The listing builds one solid part. Answer for the finished solid, in the listing's coordinates (mm). Face numbers are marked on the shaded views. A direction names the side the tool comes from. Round coordinates to 2 decimals unless told otherwise and drop trailing zeros. Write each loop counter-clockwise with the first axis right and the second up, starting at its lowest first coordinate (ties: lowest second). Pieces come first, ordered by that corner, then holes. Notation, with made-up numbers: (38, -28.75) - (63, -28.75) arc R15 cw to (63, -7.75) - close; hole circle Ø5 at (-40, 41). An arc over 180 degrees is marked (long way). Answer in a Markdown table with one row per item.
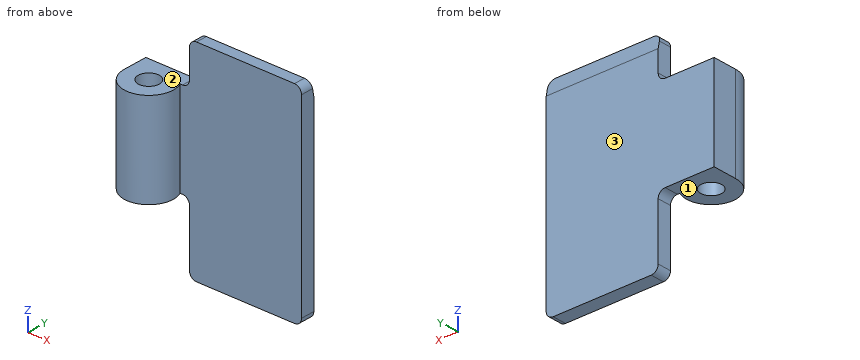
from build123d import *

# Parameters (mm, degrees)
SKETCH1_R           = 1.75
BOSS_EXTRUDE1_DEPTH = 6.7
SKETCH2_R           = 0.75
CUT_EXTRUDE1_DEPTH  = 8.142478561
SKETCH3_W           = 12
SKETCH3_H           = 6.7
BOSS_EXTRUDE2_DEPTH = 1
BOSS_EXTRUDE3_START = -6.7
BOSS_EXTRUDE3_DEPTH = 6.7
SKETCH5_W           = 8
SKETCH5_H           = 1
BOSS_EXTRUDE4_DEPTH = 3
SKETCH6_W           = 8
SKETCH6_H           = 1
BOSS_EXTRUDE5_DEPTH = 5
CHAMFER1_SIZE       = 1
CHAMFER1_SIZE2      = 0.2
FILLET1_R           = 0.5


with BuildPart() as part:
    # Sketch1 → Boss-Extrude1 (new body)
    with BuildSketch(Plane.XY):
        Circle(SKETCH1_R)
    extrude(amount=BOSS_EXTRUDE1_DEPTH)

    # Sketch2 → Cut-Extrude1 (cut, through all)
    with BuildSketch(Plane.XY.offset(6.7)):
        Circle(SKETCH2_R)
    extrude(amount=-CUT_EXTRUDE1_DEPTH, mode=Mode.SUBTRACT)

    # Sketch3 → Boss-Extrude2 (add)
    with BuildSketch(Plane(origin=(0, 1.75, 0), x_dir=(1, 0, 0), z_dir=(0, 1, 0))):
        with Locations((4.25, -3.35)):
            Rectangle(SKETCH3_W, SKETCH3_H)
    extrude(amount=-BOSS_EXTRUDE2_DEPTH)

    # Sketch4 → Boss-Extrude3 (add)
    with BuildSketch(Plane.XY.offset(6.7).offset(BOSS_EXTRUDE3_START)):
        with BuildLine():
            Line((-1.75, 0.75), (-1.75, 0))
            ThreePointArc((-1.75, 0), (-1.707262861, 0.384387205), (-1.58113883, 0.75))
            Line((-1.58113883, 0.75), (-1.75, 0.75))
        make_face()
    extrude(amount=BOSS_EXTRUDE3_DEPTH)

    # Sketch5 → Boss-Extrude4 (add)
    with BuildSketch(Plane.XY.offset(6.7)):
        with Locations((6.25, 1.25)):
            Rectangle(SKETCH5_W, SKETCH5_H)
    extrude(amount=BOSS_EXTRUDE4_DEPTH)

    # Sketch6 → Boss-Extrude5 (add)
    with BuildSketch(Plane(origin=(0, 0, 0), x_dir=(-1, 0, 0), z_dir=(0, 0, -1))):
        with Locations((-6.25, 1.25)):
            Rectangle(SKETCH6_W, SKETCH6_H)
    extrude(amount=BOSS_EXTRUDE5_DEPTH)

    # Chamfer1
    chamfer1_edges = [part.edges().sort_by_distance(p)[0] for p in [
        (6.25, 1.75, 9.7),
    ]]
    chamfer1_side = [part.faces().sort_by_distance(p)[0] for p in [
        (5.136426593, 1.75, 2.535595568),
    ]]
    chamfer(chamfer1_edges, length=CHAMFER1_SIZE, length2=CHAMFER1_SIZE2, reference=chamfer1_side[0])

    # Fillet1
    fillet1_edges = [part.edges().sort_by_distance(p)[0] for p in [
        (2.25, 1.25, 6.7),
        (10.25, 1.15, 9.7),
        (2.25, 1.25, 0),
        (10.25, 1.25, -5),
        (2.25, 1.25, -5),
        (2.25, 1.15, 9.7),
    ]]
    fillet(fillet1_edges, radius=FILLET1_R)


solid = part.part
(1) Find the intervals of material crossed by line 1 (X direction, y = 0, z = 4); line 2 (Y direction, x = 6, z = -4), in increasing order.
Checked values:
| item | result |
|---|---|
| line 1 | x = -1.75 to -0.75, 0.75 to 1.75 |
| line 2 | y = 0.75 to 1.75 |
(2) For the marked faces 1, 2 and 3, determine the directions among +Z, -Z, +X, -X, +Y, -Y from which every point of the face is accessible in a straight line to the end or side of a thin tool.
Checked values:
| item | result |
|---|---|
| face 1 | -Z, -X, +Y, -Y |
| face 2 | +Z, -X, +Y, -Y |
| face 3 | +Z, -Z, +X, -X, +Y |
(3) Flat-ended cylindrical pins translate along their axes: pin 1 (1.8 mm diameter, centred on x = 0.5, y = 0, fed in from +Z); pin 2 (4.5 mm diameter, centred on x = 8, z = 3.5, fed in from -Y); pin 3 (0.5 mm diameter, centred on y = 1, z = -2.5, fed in from -X). Find the tip coordinate at first contact, or state that the pin passes through.
Checked values:
| item | result |
|---|---|
| pin 1 | stops at z = 6.7 |
| pin 2 | stops at y = 0.75 |
| pin 3 | stops at x = 2.25 |
(4) Section A-A (x = 0) is taken. Give the vertices of the cut face in (y, z), and give its area (3 significant figures).
Checked values:
| item | result |
|---|---|
| outline | (-1.75, 0) - (-0.75, 0) - (-0.75, 6.7) - (-1.75, 6.7) - close; (0.75, 0) - (1.75, 0) - (1.75, 6.7) - (0.75, 6.7) - close |
| area | 13.4 mm2 |
(5) Section D-D (z = 8.25) is taken. Give the vertices of the cut face in (x, y).
Checked values:
| item | result |
|---|---|
| outline | (2.25, 0.75) - (10.25, 0.75) - (10.25, 1.75) - (2.25, 1.75) - close |
(6) Section C-C (z = 6.5) is taken. Give the vertices of the cut face in (x, y), and give its area (3 significant figures).
Checked values:
| item | result |
|---|---|
| outline | (-1.75, 0) arc R1.75 ccw (long way) to (1.58, 0.75) - (10.25, 0.75) - (10.25, 1.75) - (-1.75, 1.75) - close; hole circle Ø1.5 at (0, 0) |
| area | 17.6 mm2 |
(7) Section B-B (y = -0.55) is taken. Give the vertices of the cut face in (x, z), and give its area (3 significant figures).
Checked values:
| item | result |
|---|---|
| outline | (-1.66, 0) - (-0.51, 0) - (-0.51, 6.7) - (-1.66, 6.7) - close; (0.51, 0) - (1.66, 0) - (1.66, 6.7) - (0.51, 6.7) - close |
| area | 15.4 mm2 |
